The model under review builds one solid part; all positions refer to its coordinate system, in mm. Face numbers are marked on the shaded views. A direction names the side the tool comes from. Give positions to 0.01 mm unless a question says otherwise; leave off trailing zeros. Order: outer loops, then holes, each group sorted by start corner. A loop starts at its lowest first (then second) coordinate and runs counter-clockwise, first axis right, second up.
```python
from build123d import *

# Parameters (mm, degrees)
SKETCH_1_R          = 5
EXTRUDE_1_DEPTH     = 20
SKETCH_2_R          = 7.5
EXTRUDE_2_DEPTH     = 7
SKETCH_3_R          = 11
EXTRUDE_3_DEPTH     = 4.5
CHAMFER_1_SIZE      = 1
CHAMFER_2_SIZE      = 0.2
CHAMFER_3_SIZE      = 0.2
CUT_EXTRUDE_1_DEPTH = 4


with BuildPart() as part:
    # 草图1 → 凸台-拉伸1 (new body)
    with BuildSketch(Plane(origin=(0, 0, 0), x_dir=(1, 0, 0), z_dir=(0, 1, 0))):
        with Locations(Location((0, 0, 0), (0, 0, 270))):
            Circle(SKETCH_1_R)
    extrude(amount=EXTRUDE_1_DEPTH)

    # 草图2 → 凸台-拉伸2 (add)
    with BuildSketch(Plane(origin=(0, 20, 0), x_dir=(1, 0, 0), z_dir=(0, 1, 0))):
        with Locations(Location((0, 0, 0), (0, 0, 270))):
            Circle(SKETCH_2_R)
    extrude(amount=EXTRUDE_2_DEPTH)

    # 草图3 → 凸台-拉伸3 (add)
    with BuildSketch(Plane(origin=(0, 27, 0), x_dir=(1, 0, 0), z_dir=(0, 1, 0))):
        with Locations(Location((0, 0, 0), (0, 0, 270))):
            Circle(SKETCH_3_R)
    extrude(amount=EXTRUDE_3_DEPTH)

    # 倒角1
    chamfer_1_edges = [part.edges().sort_by_distance(p)[0] for p in [
        (0, 31.5, -11),
    ]]
    chamfer(chamfer_1_edges, length=CHAMFER_1_SIZE)

    # 倒角2
    chamfer_2_edges = [part.edges().sort_by_distance(p)[0] for p in [
        (0, 20, -7.5),
    ]]
    chamfer(chamfer_2_edges, length=CHAMFER_2_SIZE)

    # 倒角3
    chamfer_3_edges = [part.edges().sort_by_distance(p)[0] for p in [
        (0, 0, -5),
    ]]
    chamfer(chamfer_3_edges, length=CHAMFER_3_SIZE)

    # 草图4 → 切除-拉伸1 (cut)
    with BuildSketch(Plane(origin=(0, 31.5, 0), x_dir=(1, 0, 0), z_dir=(0, 1, 0))):
        Polygon((2.309401077, 0), (1.154700538, 2), (-1.154700538, 2), (-2.309401077, 0), (-1.154700538, -2), (1.154700538, -2), align=None)
    extrude(amount=-CUT_EXTRUDE_1_DEPTH, mode=Mode.SUBTRACT)


solid = part.part
```
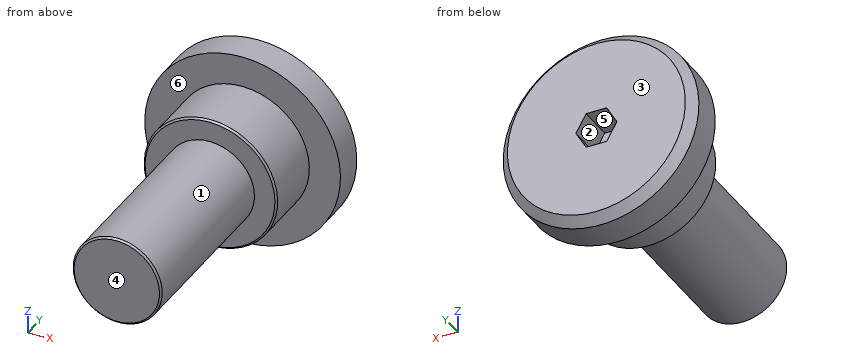
Item 1: For line 1 (Y direction, x = 2.5, z = -6); line 2 (Y direction, x = -7.75, z = 5); line 3 (Z direction, x = -1.25, y = 28.5), list the stretches that pass through material, from the lowest coordinate up.
Values found:
line 1: y = 20 to 31.5
line 2: y = 27 to 31.5
line 3: z = -10.93 to -1.83, 1.83 to 10.93
Item 2: Take a section at A-A (x = 0). Give the boundary of the cut face in (y, z).
Values found:
outline: (0, -4.8) - (0.2, -5) - (20, -5) - (20, -7.3) - (20.2, -7.5) - (27, -7.5) - (27, -11) - (30.5, -11) - (31.5, -10) - (31.5, -2) - (27.5, -2) - (27.5, 2) - (31.5, 2) - (31.5, 10) - (30.5, 11) - (27, 11) - (27, 7.5) - (20.2, 7.5) - (20, 7.3) - (20, 5) - (0.2, 5) - (0, 4.8) - close
Item 3: Draft analysis for pull direction Z (two halves, no side actions). For the marked faces 1, 2 and 3, state which applies: released by +Z, released by -Z, zero draft, split by the parting line, or undercut.
Values found:
face 1: split by the parting line
face 2: undercut
face 3: zero draft
Item 4: Take a section at B-B (y = 2). Give the boundary of the cut face in (x, z).
Values found:
outline: circle Ø10 at (0, 0)
Item 5: Clearance check with flat-ended pins moving along their axes: pin 1 Ø10 at (x, y) = (3.5, 3) entering from +Z; pin 2 Ø1.2 at (x, z) = (1, -0.5) entering from +Y; pin 3 Ø4 at (y, z) = (11, -1.5) entering from -X; pin 4 Ø5 at (x, y) = (-8.5, 6) entering from -Z. State where each tip first meets the part, or that it passes through.
Values found:
pin 1: stops at z = 5
pin 2: stops at y = 27.5
pin 3: stops at x = -5
pin 4: passes through
Item 6: For the marked faces 4, 5 and 6, list the 3-axis set-ups (+Z, -Z, +X, -X, +Y, -Y) from which the entire face can be reached by the end or side of a thin tool; tool diameter is ignored.
Values found:
face 4: +Z, -Z, +X, -X, -Y
face 5: +Y
face 6: -Y
